Geometry check sheet. Reference: the model listing, model coordinates, mm. Give positions to 0.01 mm unless a question says otherwise; leave off trailing zeros. Loops run counter-clockwise (first coordinate to the right, second up) from the corner with the lowest first, then second, coordinate; pieces in that order, holes last. Notation, with made-up numbers: (-38, -14) -> (-18, -14) arc R31 cw to (-18, 24) -> close; hole circle Ø11 at (-10, 44). An arc over 180 degrees is marked (long way). Write item = value, one per line. Start each with the question number.
```python
from build123d import *

# Parameters (mm, degrees)
SKETCH1_R           = 12.5
BOSS_EXTRUDE1_DEPTH = 1530
CUT_EXTRUDE1_START  = -11
SKETCH_2_2_W        = 44.374102045
SKETCH_2_2_H        = 48.77153558
SKETCH_2_2_W_2      = 134.556182266
SKETCH_2_2_H_2      = 57.966169337
CUT_EXTRUDE1_DEPTH  = 20
CUT_EXTRUDE2_START  = 11
SKETCH_2_2_2_W      = 44.374102045
SKETCH_2_2_2_H      = 48.77153558
SKETCH_2_2_2_W_2    = 134.556182266
SKETCH_2_2_2_H_2    = 57.966169337
CUT_EXTRUDE2_DEPTH  = 20


with BuildPart() as part:
    # Sketch1 → Boss-Extrude1 (new body)
    with BuildSketch(Plane(origin=(0, 0, 0), x_dir=(0, 0, -1), z_dir=(1, 0, 0))):
        Circle(SKETCH1_R)
    extrude(amount=BOSS_EXTRUDE1_DEPTH)

    # Sketch 2_2 → Cut-Extrude1 (cut)
    with BuildSketch(Plane.XY.offset(CUT_EXTRUDE1_START)):
        with Locations((13.812948977, 5.596733591)):
            Rectangle(SKETCH_2_2_W, SKETCH_2_2_H)
        with Locations((1561.278091133, 0.999416713)):
            Rectangle(SKETCH_2_2_W_2, SKETCH_2_2_H_2)
    extrude(amount=-CUT_EXTRUDE1_DEPTH, mode=Mode.SUBTRACT)

    # Sketch 2_2 2 → Cut-Extrude2 (cut)
    with BuildSketch(Plane.XY.offset(CUT_EXTRUDE2_START)):
        with Locations((13.812948977, 5.596733591)):
            Rectangle(SKETCH_2_2_2_W, SKETCH_2_2_2_H)
        with Locations((1561.278091133, 0.999416713)):
            Rectangle(SKETCH_2_2_2_W_2, SKETCH_2_2_2_H_2)
    extrude(amount=CUT_EXTRUDE2_DEPTH, mode=Mode.SUBTRACT)


solid = part.part
```
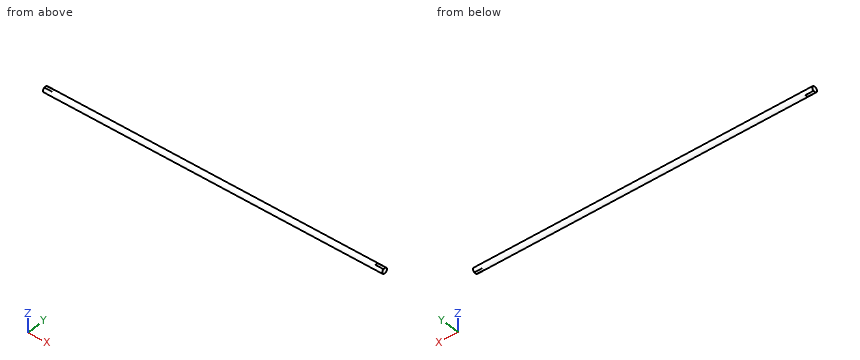
1) Thickness scan on line 1 (Z direction, x = 331, y = 6.25); line 2 (Y direction, x = 802.5, z = -5.75); line 3 (Z direction, x = 493, y = -5.5). Record the ranges inside material, lowest first.
2) Section check A-A (x = 1245). Enter the section's corners in (y, z), plus the area to 3 significant figures.
3) Section check B-B (z = 6.5). Enter the section's corners in (x, y), plus the area to 3 significant figures.
4) Depth check by flat-ended pin: pin 1 Ø9.5 at (x, y) = (10, 1.5) entering from +Z; pin 2 Ø0.5 at (y, z) = (-0.5, -12) entering from -X; pin 3 Ø6 at (x, y) = (24.5, 1.5) entering from -Z; pin 4 Ø3 at (y, z) = (-2.5, 9) entering from -X. Enter the tip coordinate at first touch or a pass-through.
Check result:
q1.line_1 = -10.83 to 10.83
q1.line_2 = -11.1 to 11.1
q1.line_3 = -11.22 to 11.22
q2.outline = circle Ø25 at (0, 0)
q2.area = 491 mm2
q3.outline = (0, -10.68) -> (1530, -10.68) -> (1530, 10.68) -> (0, 10.68) -> close
q3.area = 32,700 mm2
q4.pin_1 = 11
q4.pin_2 = 36
q4.pin_3 = -11
q4.pin_4 = 0
